The listing builds one solid part. Answer for the finished solid, in the listing's coordinates (mm). Face numbers are marked on the shaded views. A direction names the side the tool comes from. Round coordinates to 2 decimals unless told otherwise and drop trailing zeros. Loops run counter-clockwise (first coordinate to the right, second up) from the corner with the lowest first, then second, coordinate; pieces in that order, holes last. Notation, with made-up numbers: (79.25, 15.25) -> (102.25, 15.25) arc R15 ccw to (102.25, 21.25) -> close; hole circle Ø8 at (4, -1.5). An arc over 180 degrees is marked (long way). One line per question, with ' | ' between items.
from build123d import *

# Parameters (mm, degrees)
SKETCH1_R           = 3
SKETCH1_W           = 8
SKETCH1_H           = 110
BOSS_EXTRUDE1_DEPTH = 10


with BuildPart() as part:
    # Sketch1 → Boss-Extrude1 (new body)
    with BuildSketch(Plane.XY):
        with BuildLine():
            Line((2.118738771, -10.491083349), (0, 0))
            Line((0, 0), (0, 120))
            Line((0, 120), (2.092997217, 131.74896535))
            ThreePointArc((2.092997217, 131.74896535), (8, 136.696673509), (13.907002783, 131.74896535))
            Line((13.907002783, 131.74896535), (16, 120))
            Line((16, 120), (16, 0))
            Line((16, 0), (13.881261229, -10.491083349))
            ThreePointArc((13.881261229, -10.491083349), (8, -15.303326491), (2.118738771, -10.491083349))
        make_face()
        with Locations((8, 130.696673509)):
            Circle(SKETCH1_R, mode=Mode.SUBTRACT)
        with Locations((8, -9.303326491)):
            Circle(SKETCH1_R, mode=Mode.SUBTRACT)
        with Locations((8, 60)):
            Rectangle(SKETCH1_W, SKETCH1_H, mode=Mode.SUBTRACT)
    extrude(amount=BOSS_EXTRUDE1_DEPTH)


solid = part.part
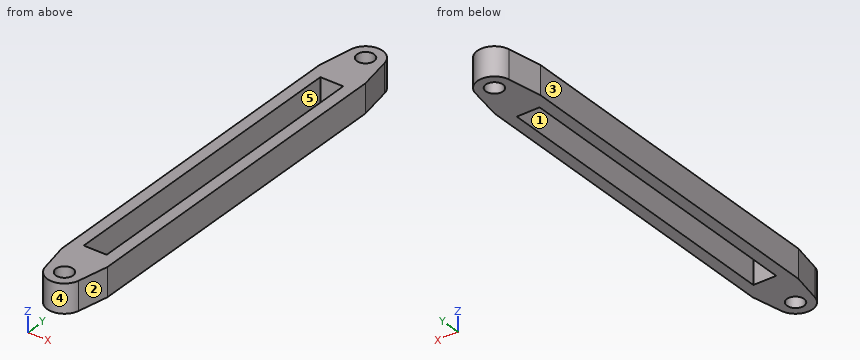
Q1. A cutting plane is placed at A-A on x = 8. Give the vertices of the cut face in (y, z), plus the area to 3 significant figures.
Numbers:
outline: (-15.3, 0) -> (-12.3, 0) -> (-12.3, 10) -> (-15.3, 10) -> close; (-6.3, 0) -> (5, 0) -> (5, 10) -> (-6.3, 10) -> close; (115, 0) -> (127.7, 0) -> (127.7, 10) -> (115, 10) -> close; (133.7, 0) -> (136.7, 0) -> (136.7, 10) -> (133.7, 10) -> close | area: 300 mm^2
Q2. For the marked faces 1 and 2, determine the directions among +Z, -Z, +X, -X, +Y, -Y from which every point of the face is accessible in a straight line to the end or side of a thin tool.
Numbers:
face 1: +Z, -Z | face 2: +Z, -Z, +X, -Y
Q3. Find the intervals of material crossed by line 1 (X direction, y = 37, z = 2); line 2 (Y direction, x = 9.25, z = 8.5); line 3 (Y direction, x = 7.5, z = 3.75), in increasing order. Write a range as from..to.
Numbers:
line 1: 0..4, 12..16 | line 2: -15.17..-12.03, -6.58..5, 115..127.97, 133.42..136.57 | line 3: -15.28..-12.26, -6.35..5, 115..127.74, 133.65..136.68
Q4. For a pull along Y with two mould halves and no side action, classify the marked faces 3, 4 and 5 as pulls with the +Y half, pulls with the -Y half, needs draft (parallel to the pull), parting line crosses it, or undercut.
Numbers:
face 3: needs draft | face 4: pulls with the -Y half | face 5: undercut
Q5. A cutting plane is placed at B-B on y = 90.5. Give the vertices of the cut face in (x, z).
Numbers:
outline: (0, 0) -> (4, 0) -> (4, 10) -> (0, 10) -> close; (12, 0) -> (16, 0) -> (16, 10) -> (12, 10) -> close
Q6. A cutting plane is placed at C-C on z = 6. Give the vertices of the cut face in (x, y).
Numbers:
outline: (0, 0) -> (2.12, -10.49) arc R6 ccw to (13.88, -10.49) -> (16, 0) -> (16, 120) -> (13.91, 131.75) arc R6 ccw to (2.09, 131.75) -> (0, 120) -> close; hole (4, 5) -> (12, 5) -> (12, 115) -> (4, 115) -> close; hole circle Ø6 at (8, -9.3); hole circle Ø6 at (8, 130.7)
Q7. Given pin 1 Ø1 at (x, z) = (5.5, 3.5) entering from -Y, flat-ended and moving along its own axis, determine where the tip first touches the part or whether it passes through.
Numbers:
pin 1: y = -14.96
